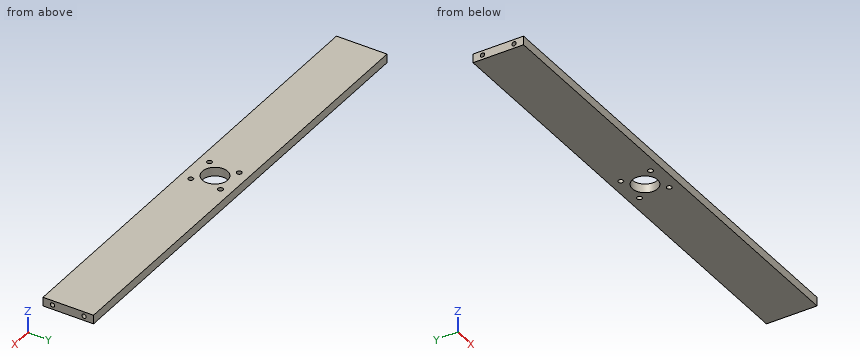
from build123d import *

# Parameters (mm, degrees)
SKETCH1_W             = 735
SKETCH1_H             = 80
BOSS_EXTRUDE1_DEPTH   = 14
SKETCH2_R             = 4
SKETCH2_R_2           = 20
CUT_EXTRUDE1_DEPTH    = 14
M8_TAPPED_HOLE1_D     = 6.8
M8_TAPPED_HOLE1_DEPTH = 19.75
M8_TAPPED_HOLE1_TIP   = 2.042926105
M8_TAPPED_HOLE2_D     = 6.8
M8_TAPPED_HOLE2_DEPTH = 19.75
M8_TAPPED_HOLE2_TIP   = 2.042926105


with BuildPart() as part:
    # Sketch1 → Boss-Extrude1 (new body)
    with BuildSketch(Plane.XY):
        with Locations((367.5, 40)):
            Rectangle(SKETCH1_W, SKETCH1_H)
    extrude(amount=BOSS_EXTRUDE1_DEPTH)

    # Sketch2 → Cut-Extrude1 (cut)
    with BuildSketch(Plane.XY.offset(14)):
        with Locations((344, 63.5)):
            Circle(SKETCH2_R)
        with Locations((344, 16.5)):
            Circle(SKETCH2_R)
        with Locations((391, 16.5)):
            Circle(SKETCH2_R)
        with Locations((391, 63.5)):
            Circle(SKETCH2_R)
        with Locations((367.5, 40)):
            Circle(SKETCH2_R_2)
    extrude(amount=-CUT_EXTRUDE1_DEPTH, mode=Mode.SUBTRACT)

    # M8 Tapped Hole1
    with Locations(Plane(origin=(0, 65, 7), x_dir=(0, 0, -1), z_dir=(-1, 0, 0))):
        with Locations((0, 0), (0, 50)):
            Hole(M8_TAPPED_HOLE1_D / 2, depth=M8_TAPPED_HOLE1_DEPTH)
            with Locations((0, 0, -(M8_TAPPED_HOLE1_DEPTH + M8_TAPPED_HOLE1_TIP / 2))):  # 118° drill point
                Cone(0, M8_TAPPED_HOLE1_D / 2, M8_TAPPED_HOLE1_TIP, mode=Mode.SUBTRACT)

    # M8 Tapped Hole2
    with Locations(Plane(origin=(735, 15, 7), x_dir=(0, 0, 1), z_dir=(1, 0, 0))):
        with Locations((0, 0), (0, -50)):
            Hole(M8_TAPPED_HOLE2_D / 2, depth=M8_TAPPED_HOLE2_DEPTH)
            with Locations((0, 0, -(M8_TAPPED_HOLE2_DEPTH + M8_TAPPED_HOLE2_TIP / 2))):  # 118° drill point
                Cone(0, M8_TAPPED_HOLE2_D / 2, M8_TAPPED_HOLE2_TIP, mode=Mode.SUBTRACT)


solid = part.part
The model under review builds one solid part; all positions refer to its coordinate system, in mm. Give positions to 0.01 mm unless a question says otherwise; leave off trailing zeros. Write each loop counter-clockwise with the first axis right and the second up, starting at its lowest first coordinate (ties: lowest second). Pieces come first, ordered by that corner, then holes.
1. Wall thickness on L1, parallel to Y at x = 723, z = 7; L2, parallel to Y at x = 344, z = 4.75; L3, parallel to Z at x = 8.25, y = 15: over which ranges is each line inside the solid? List them lowest first.
2. Add section A-A, the plane y = 40. Write out the cut boundary in (x, z).
3. For P1, Ø6, axis at y = 65, z = 7, coming from the -X side; P2, Ø4, axis at y = 65, z = 7, coming from the +X side; P3, Ø5.5, axis at y = 15, z = 7, coming from the +X side, all flat-tipped, find the tip position at first contact; note any pin that passes through.
Worked answers:
1. L1: y = 0 to 11.6, 18.4 to 61.6, 68.4 to 80
1. L2: y = 0 to 12.5, 20.5 to 59.5, 67.5 to 80
1. L3: z = 0 to 3.6, 10.4 to 14
2. outline: (0, 0) - (347.5, 0) - (347.5, 14) - (0, 14) - close; (387.5, 0) - (735, 0) - (735, 14) - (387.5, 14) - close
3. P1: stops at x = 19.99
3. P2: stops at x = 714.41
3. P3: stops at x = 714.86
